Source: CAD feature listing. Evaluate the final solid. Frame: model axes, mm. Face numbers are marked on the shaded views. Round coordinates to 2 decimals unless told otherwise and drop trailing zeros. Write each loop counter-clockwise with the first axis right and the second up, starting at its lowest first coordinate (ties: lowest second). Pieces come first, ordered by that corner, then holes. Notation, with made-up numbers: (28.25, 66) -> (33.25, 66) arc R22 ccw to (33.25, 102) -> close; hole circle Ø4 at (88.5, -18.5). An arc over 180 degrees is marked (long way). Return JSON: item names as keys, results as strings. Group by question number.
from build123d import *

# Parameters (mm, degrees)
SKETCH1_W           = 26
SKETCH1_H           = 15
SKETCH1_R           = 3
BOSS_EXTRUDE1_DEPTH = 20
SKETCH2_R           = 5
CUT_EXTRUDE1_DEPTH  = 34.648922717


with BuildPart() as part:
    # Sketch1 → Boss-Extrude1 (new body)
    with BuildSketch(Plane.XY):
        Rectangle(SKETCH1_W, SKETCH1_H)
        Circle(SKETCH1_R, mode=Mode.SUBTRACT)
    extrude(amount=BOSS_EXTRUDE1_DEPTH)

    # Sketch2 → Cut-Extrude1 (cut, through all)
    with BuildSketch(Plane(origin=(13, 0, 0), x_dir=(0, 0, -1), z_dir=(1, 0, 0))):
        with Locations((-10, 0)):
            Circle(SKETCH2_R)
    extrude(amount=-CUT_EXTRUDE1_DEPTH, mode=Mode.SUBTRACT)


solid = part.part
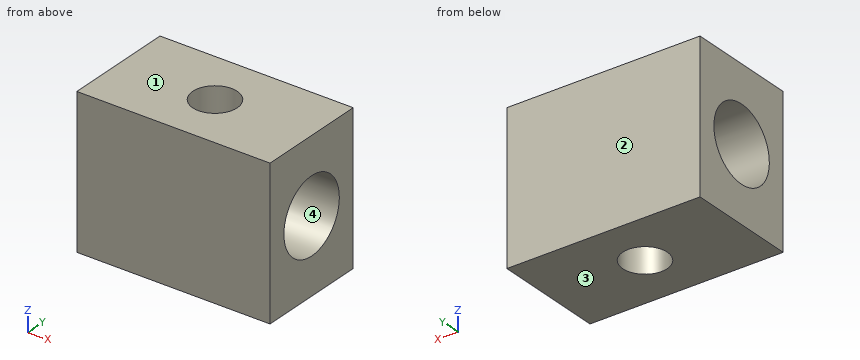
Item 1: Pull-direction query (Z, two-part tool) for the marked faces 1, 2, 3 and 4; classes: +Z half, -Z half, draft (parallel to the pull), parting line (faces both ways), or undercut.
Item 2: Cut plane A-A on x = 0. Output: boundary loops of the cut face in (y, z), and give its area (3 significant figures).
Item 3: Cut plane C-C on y = -1.25. Output: boundary loops of the cut face in (x, z).
Item 4: First-contact query: pin 1 Ø8 at (y, z) = (-1.5, 14) entering from -X. Flat tip, straight axial feed; report the tip coordinate or a pass-through.
Item 5: Material intervals for probe 1 along Y at (x, z) = (-5.5, 9.75); probe 2 along X at (y, z) = (0, 2.75); probe 3 along Y at (x, z) = (0, 17.5), sorted ascending.
Item 6: Cut plane D-D on z = 17.5. Output: boundary loops of the cut face in (x, y), and give its area (3 significant figures).
Item 7: Cut plane B-B on z = 10. Output: boundary loops of the cut face in (x, y).
Here are the results:
{
 "1": {"face 1": "+Z half", "face 2": "draft", "face 3": "-Z half", "face 4": "undercut"},
 "2": {"outline": "(-7.5, 0) -> (-3, 0) -> (-3, 6) arc R5 cw to (-3, 14) -> (-3, 20) -> (-7.5, 20) -> close; (3, 0) -> (7.5, 0) -> (7.5, 20) -> (3, 20) -> (3, 14) arc R5 cw to (3, 6) -> close", "area": "158 mm^2"},
 "3": {"outline": "(-13, 0) -> (-2.73, 0) -> (-2.73, 5.16) -> (-13, 5.16) -> close; (-13, 14.84) -> (-2.73, 14.84) -> (-2.73, 20) -> (-13, 20) -> close; (2.73, 0) -> (13, 0) -> (13, 5.16) -> (2.73, 5.16) -> close; (2.73, 14.84) -> (13, 14.84) -> (13, 20) -> (2.73, 20) -> close"},
 "4": {"pin 1": "stops at x = -13"},
 "5": {"probe 1": "y = -7.5 to -4.99, 4.99 to 7.5", "probe 2": "x = -13 to -3, 3 to 13", "probe 3": "y = -7.5 to -3, 3 to 7.5"},
 "6": {"outline": "(-13, -7.5) -> (13, -7.5) -> (13, 7.5) -> (-13, 7.5) -> close; hole circle Ø6 at (0, 0)", "area": "362 mm^2"},
 "7": {"outline": "(-13, -7.5) -> (13, -7.5) -> (13, -5) -> (-13, -5) -> close; (-13, 5) -> (13, 5) -> (13, 7.5) -> (-13, 7.5) -> close"}
}
